Job drawing, mm, ordinate dimensions from the low corner. One solid piece. Give positions to 0.01 mm unless a question says otherwise; leave off trailing zeros. Write each loop counter-clockwise with the first axis right and the second up, starting at its lowest first coordinate (ties: lowest second). Pieces come first, ordered by that corner, then holes. Notation, with made-up numbers: M 15,23.25 L 48,23.25 A3 cw 48,27.25 Z; hole C 79,54.5 d9. An arc over 180 degrees is marked long. Use a Markdown table: item, result.
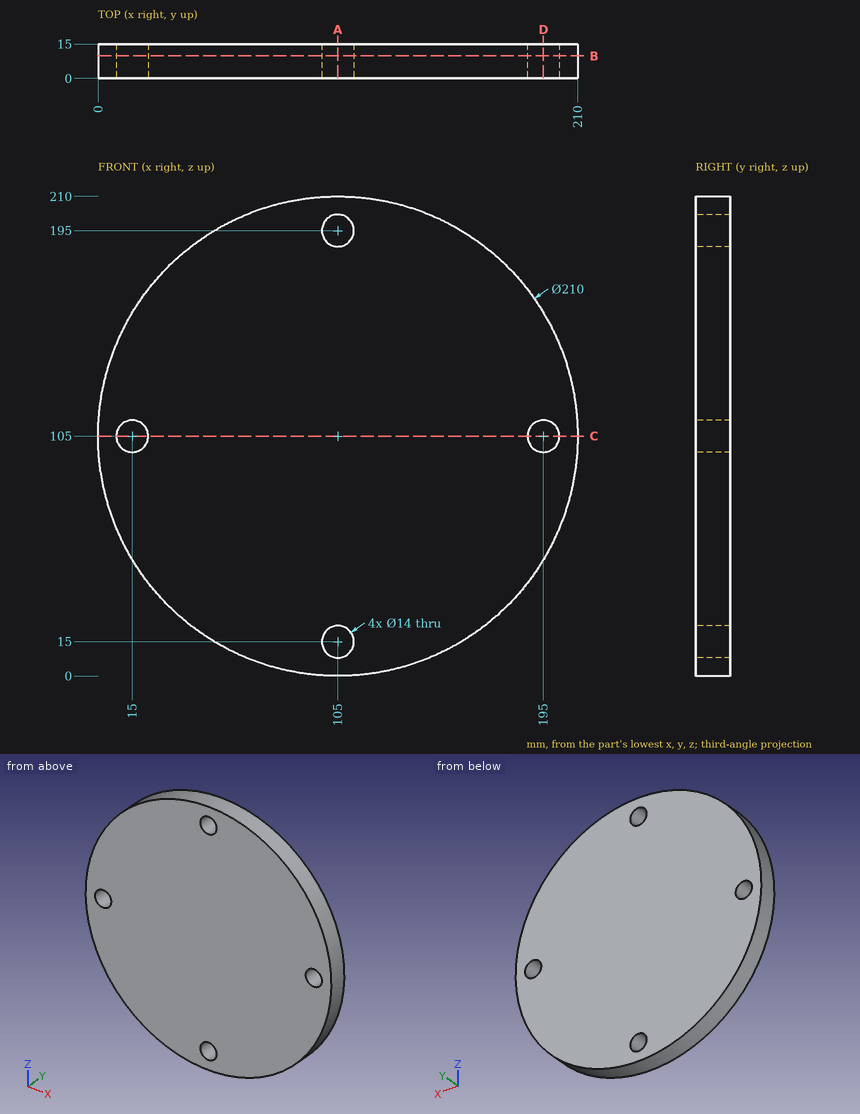
1. Drop flat-ended pins along their axis: P1, Ø3, axis at x = 97, y = 6, coming from the +Z side; P2, Ø6, axis at x = 156.5, y = 1.5, coming from the -Z side; P3, Ø8, axis at y = 2.5, z = 165.5, coming from the +X side; P4, Ø2, axis at x = 22, z = 160, coming from the -Y side. Give the stop position or say it passes through.
Findings below:
| item | result |
|---|---|
| P1 | z = 209.8 |
| P2 | z = 11.87 |
| P3 | x = 193.5 |
| P4 | y = 0 |
2. Cut at B-B, the plane y = 9.75. Give the cut face in (x, z).
Findings below:
| item | result |
|---|---|
| outline | C 105,105 d210; hole C 15,105 d14; hole C 105,15 d14; hole C 105,195 d14; hole C 195,105 d14 |
3. Drill centre lines: L1, parallel to X at y = 4.75, z = 105; L2, parallel to Z at x = 195, y = 7.5. Where is each one in solid material? Low to high.
Findings below:
| item | result |
|---|---|
| L1 | 0 to 8, 22 to 188, 202 to 210 |
| L2 | 50.92 to 98, 112 to 159.08 |
4. Cut at C-C, the plane z = 105. Give the cut face in (x, y), then the cut area to 3 significant figures.
Findings below:
| item | result |
|---|---|
| outline | M 0,0 L 8,0 L 8,15 L 0,15 Z; M 22,0 L 188,0 L 188,15 L 22,15 Z; M 202,0 L 210,0 L 210,15 L 202,15 Z |
| area | 2,730 mm2 |
5. Cut at A-A, the plane x = 105. Give the cut face in (y, z).
Findings below:
| item | result |
|---|---|
| outline | M 0,0 L 15,0 L 15,8 L 0,8 Z; M 0,22 L 15,22 L 15,188 L 0,188 Z; M 0,202 L 15,202 L 15,210 L 0,210 Z |
6. Cut at D-D, the plane x = 195. Give the cut face in (y, z).
Findings below:
| item | result |
|---|---|
| outline | M 0,50.92 L 15,50.92 L 15,98 L 0,98 Z; M 0,112 L 15,112 L 15,159.08 L 0,159.08 Z |
